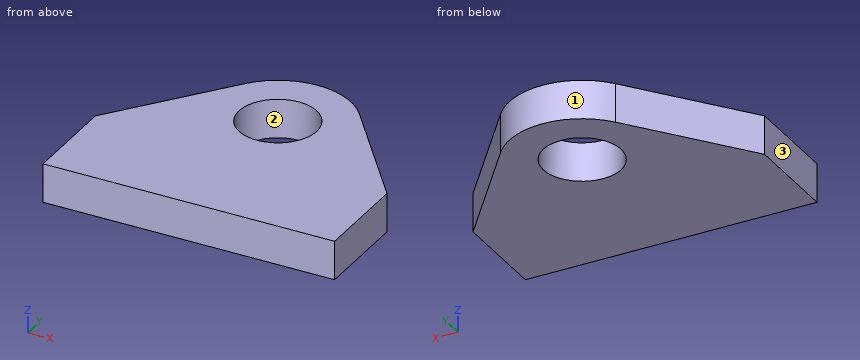
from build123d import *

# Parameters (mm, degrees)
SKETCH1_R           = 8
BOSS_EXTRUDE1_DEPTH = 8


with BuildPart() as part:
    # Sketch1 → Boss-Extrude1 (new body)
    with BuildSketch(Plane.XY):
        with BuildLine():
            Line((0, 0), (0, 20))
            Line((0, 20), (18.18643347, 43.243356849))
            ThreePointArc((18.18643347, 43.243356849), (30, 49), (41.81356653, 43.243356849))
            Line((41.81356653, 43.243356849), (60, 20))
            Line((60, 20), (60, 0))
            Line((60, 0), (0, 0))
        make_face()
        with Locations((30, 34)):
            Circle(SKETCH1_R, mode=Mode.SUBTRACT)
    extrude(amount=BOSS_EXTRUDE1_DEPTH)


solid = part.part
Check sheet for the modelled part. Datum: model origin and axes. Units: mm. Face numbers are marked on the shaded views. Round coordinates to 2 decimals unless told otherwise and drop trailing zeros. Order: outer loops, then holes, each group sorted by start corner. A loop starts at its lowest first (then second) coordinate and runs counter-clockwise, first axis right, second up.
(1) Go/stop test with a flat-tipped pin: P1, Ø4, axis at y = 31.5, z = 2, coming from the +X side. Record where the tip stops, or that it passes through.
(2) Cross-section at B-B, the plane x = 30. Enter the section's corners in (y, z).
(3) Draft check along X on the marked faces 1, 2 and 3. Enter one of: pulls with the +X half, pulls with the -X half, needs draft (parallel to the pull), parting line crosses it, or undercut.
(4) Cross-section at D-D, the plane x = 13. Enter the section's corners in (y, z).
(5) Cross-section at A-A, the plane z = 4.25. Enter the section's corners in (x, y), and give its area (3 significant figures).
(6) Scan lines: probe 1 along Y at (x, z) = (30, 4); probe 2 along X at (y, z) = (37, 7); probe 3 along Y at (x, z) = (25, 3.25) (3 decimals). Record each from-to range of solid material in increasing order.
(7) Cross-section at C-C, the plane y = 27.5. Enter the section's corners in (x, z), and give its area (3 significant figures).
Check sheet entries:
1. P1: stops at x = 52.57
2. outline: (0, 0) - (26, 0) - (26, 8) - (0, 8) - close; (42, 0) - (49, 0) - (49, 8) - (42, 8) - close
3. face 1: parting line crosses it
3. face 2: undercut
3. face 3: pulls with the -X half
4. outline: (0, 0) - (36.61, 0) - (36.61, 8) - (0, 8) - close
5. outline: (0, 0) - (60, 0) - (60, 20) - (41.81, 43.24) arc R15 ccw to (18.19, 43.24) - (0, 20) - close; hole circle Ø16 at (30, 34)
5. area: 2,070 mm2
6. probe 1: y = 0 to 26, 42 to 49
6. probe 2: x = 13.3 to 22.58, 37.42 to 46.7
6. probe 3: y = 0 to 27.755, 40.245 to 48.142
7. outline: (5.87, 0) - (25.34, 0) - (25.34, 8) - (5.87, 8) - close; (34.66, 0) - (54.13, 0) - (54.13, 8) - (34.66, 8) - close
7. area: 311 mm2
